Design review of the part built by this model. Coordinates are the model's own, in mm. A direction names the side the tool comes from. Round coordinates to 2 decimals unless told otherwise and drop trailing zeros. Loops run counter-clockwise (first coordinate to the right, second up) from the corner with the lowest first, then second, coordinate; pieces in that order, holes last. Notation, with made-up numbers: (61, -30) - (116, -30) arc R9 cw to (116, -14) - close; hole circle Ø1 at (-36.75, 53). An arc over 180 degrees is marked (long way). Return JSON: item names as keys, results as strings. Group by question number.
from build123d import *

# Parameters (mm, degrees)
SKETCH1_W           = 800
SKETCH1_H           = 400
BOSS_EXTRUDE1_DEPTH = 15
DRAFT1_ANGLE        = 1
FILLET1_R           = 10
CUT_EXTRUDE1_DEPTH  = 900
CUT_EXTRUDE2_DEPTH  = 10
FILLET2_R           = 2
SKETCH4_W           = 250
SKETCH4_H           = 15
BOSS_EXTRUDE2_DEPTH = 25
CUT_EXTRUDE4_DEPTH  = 10
SKETCH8_W           = 87.746039113
SKETCH8_H           = 29.522031851
BOSS_EXTRUDE3_DEPTH = 25
SKETCH9_R           = 5
CUT_EXTRUDE5_DEPTH  = 700


with BuildPart() as part:
    # Sketch1 → Boss-Extrude1 (new body)
    with BuildSketch(Plane(origin=(0, 0, 0), x_dir=(1, 0, 0), z_dir=(0, 1, 0))):
        Rectangle(SKETCH1_W, SKETCH1_H)
    extrude(amount=-BOSS_EXTRUDE1_DEPTH)

    # Draft1
    draft1_faces = [part.faces().sort_by_distance(p)[0] for p in [
        (0, -7.5, 200),
    ]]
    draft(draft1_faces, Plane(origin=(0, -15, 0), x_dir=(0, 0, -1), z_dir=(0, -1, 0)), DRAFT1_ANGLE)

    # Fillet1
    fillet1_edges = [part.edges().sort_by_distance(p)[0] for p in [
        (400, -7.5, 200.130912987),
        (-400, -7.5, 200.130912987),
        (-400, -7.5, -200),
        (400, -7.5, -200),
    ]]
    fillet(fillet1_edges, radius=FILLET1_R)

    # Sketch2 → Cut-Extrude1 (cut)
    with BuildSketch(Plane.ZY.offset(400)):
        Polygon((185.261825974, 0), (200.130912987, -7.5), (200.261825974, 0), align=None)
    extrude(amount=-CUT_EXTRUDE1_DEPTH, mode=Mode.SUBTRACT)

    # Sketch3 → Cut-Extrude2 (cut)
    with BuildSketch(Plane(origin=(0, 0, 0), x_dir=(1, 0, 0), z_dir=(0, 1, 0))):
        with BuildLine():
            Line((-150, -130), (150, -130))
            ThreePointArc((150, -130), (170, -150), (150, -170))
            Line((150, -170), (-150, -170))
            ThreePointArc((-150, -170), (-170, -150), (-150, -130))
        make_face()
    extrude(amount=-CUT_EXTRUDE2_DEPTH, mode=Mode.SUBTRACT)

    # Fillet2
    fillet2_edges = [part.edges().sort_by_distance(p)[0] for p in [
        (-170, -10, 150),
        (0, -10, 130),
        (170, -10, 150),
        (0, -10, 170),
        (-170, 0, 150),
        (0, 0, 170),
        (170, 0, 150),
        (0, 0, 130),
    ]]
    fillet(fillet2_edges, radius=FILLET2_R)

    # Sketch4 → Boss-Extrude2 (add)
    with BuildSketch(Plane.XZ.offset(15)):
        with Locations((-230, 66.25)):
            Rectangle(SKETCH4_W, SKETCH4_H)
    boss_extrude2 = extrude(amount=BOSS_EXTRUDE2_DEPTH)

    # Sketch7 → Cut-Extrude4 (cut)
    with BuildSketch(Plane(origin=(0, 0, 58.75), x_dir=(-1, 0, 0), z_dir=(0, 0, -1))):
        with BuildLine():
            Line((335, -33.5), (125, -33.5))
            ThreePointArc((125, -33.5), (119, -27.5), (125, -21.5))
            Line((125, -21.5), (335, -21.5))
            ThreePointArc((335, -21.5), (341, -27.5), (335, -33.5))
        make_face()
    cut_extrude4 = extrude(amount=-CUT_EXTRUDE4_DEPTH, mode=Mode.SUBTRACT)

    # Mirror2: Boss-Extrude2, Cut-Extrude4 across plane
    add(boss_extrude2.mirror(Plane.XY.offset(-36.25)))
    add(cut_extrude4.mirror(Plane.XY.offset(-36.25)), mode=Mode.SUBTRACT)

    # Sketch8 → Boss-Extrude3 (add)
    with BuildSketch(Plane.XZ.offset(15)):
        with Locations((310.696102603, 94.974826804)):
            Rectangle(SKETCH8_W, SKETCH8_H)
    boss_extrude3 = extrude(amount=BOSS_EXTRUDE3_DEPTH)

    # Mirror3: Boss-Extrude3 across plane
    add(boss_extrude3.mirror(Plane(origin=(0, 0, -36), x_dir=(1, 0, 0), z_dir=(0, 0, -1))))

    # Sketch9 → Cut-Extrude5 (cut)
    with BuildSketch(Plane(origin=(0, 0, -181.735842729), x_dir=(-1, 0, 0), z_dir=(0, 0, -1))):
        with Locations((-344.56912216, -27.5)):
            Circle(SKETCH9_R)
    extrude(amount=-CUT_EXTRUDE5_DEPTH, mode=Mode.SUBTRACT)


solid = part.part
Q1. Tool access review of faces 5 (the flat face through (310, -27, 109.736)), 6 (the flat face through (266.823, -27, 95)), 7 (the flat face through (-105, -27, 66)), 8 (the cylindrical face through (-170, -5, 150)): name each direction out of +Z, -Z, +X, -X, +Y, -Y from which nothing blocks a thin tool from reaching the whole face with its end or side.
Q2. Draft analysis for pull direction Z (two halves, no side actions). For faces 1 (the flat face through (2, -10, 150)), 2 (the flat face through (-232, -19, 58.75)), 3 (the flat face through (354.569, -27, -167)), 4 (the flat face through (-5.6, -3.7, 192.6)), state which applies: pulls with the +Z half, pulls with the -Z half, needs draft (parallel to the pull), parting line crosses it, or undercut.
Q3. For line 1 (X direction, y = -28.5, z = -171); line 2 (Z direction, x = 285.5, y = -25); line 3 (Z direction, x = -354.5, y = -35), list the stretches that pass through material, from the lowest coordinate up.
Q4. Add section A-A, the plane x = -322. State the section outline as (y, z) points.
Q5. Add section C-C, the plane x = 38.5. State the section outline as (y, z) points.
Q6. Insertion check: pin 1 Ø9 at (x, y) = (344.57, -27.5) entering from +Z; pin 2 Ø1 at (x, z) = (83.5, -6) entering from -Y; pin 3 Ø20 at (x, y) = (-240, -25.5) entering from +Z; pin 4 Ø7.5 at (x, y) = (319.5, -24) entering from -Z. Each pin has a flat end and moves straight along its axis. Give the tip position at first contact, or say it passes through.
Q7. Add section D-D, the plane z = 17.5. State the section outline as (x, y) points, plus the area to 3 significant figures.
Q8. Add section B-B, the plane z = 150. State the section outline as (x, y) points, plus the area to 3 significant figures.
Evaluation:
{
 "1": {"face 5": "+Z, +X, -X, -Y", "face 6": "+Z, -Z, -X, -Y", "face 7": "+Z, -Z, +X, -Y", "face 8": "+Y"},
 "2": {"face 1": "undercut", "face 2": "undercut", "face 3": "needs draft", "face 4": "pulls with the +Z half"},
 "3": {"line 1": "266.82 to 339.67, 349.47 to 354.57", "line 2": "-181.74 to -152.21, 80.21 to 109.74", "line 3": "-146.25 to -131.25, 58.75 to 73.75"},
 "4": {"outline": "(-40, -146.25) - (-15, -146.25) - (-15, -200) - (0, -200) - (0, 185.26) - (-7.5, 200.13) - (-15, 200) - (-15, 73.75) - (-40, 73.75) - (-40, 58.75) - (-33.5, 58.75) - (-33.5, 68.75) - (-21.5, 68.75) - (-21.5, 58.75) - (-15, 58.75) - (-15, -131.25) - (-21.5, -131.25) - (-21.5, -141.25) - (-33.5, -141.25) - (-33.5, -131.25) - (-40, -131.25) - close"},
 "5": {"outline": "(-15, -200) - (0, -200) - (0, 128) arc R2 ccw to (-2, 130) - (-8, 130) arc R2 cw to (-10, 132) - (-10, 168) arc R2 cw to (-8, 170) - (-2, 170) arc R2 ccw to (0, 172) - (0, 185.26) - (-7.5, 200.13) - (-15, 200) - close"},
 "6": {"pin 1": "through", "pin 2": "y = -15", "pin 3": "z = 73.75", "pin 4": "z = -181.74"},
 "7": {"outline": "(-400, -15) - (400, -15) - (400, 0) - (-400, 0) - close", "area": "12,000 mm²"},
 "8": {"outline": "(-400, -15) - (400, -15) - (400, 0) - (172, 0) arc R2 ccw to (170, -2) - (170, -8) arc R2 cw to (168, -10) - (-168, -10) arc R2 cw to (-170, -8) - (-170, -2) arc R2 ccw to (-172, 0) - (-400, 0) - close", "area": "8,600 mm²"}
}
